For this review, take the finished solid that the model builds, in its own axes (mm). Coordinates: 2 decimals unless noted, no trailing zeros. Loops run counter-clockwise (first coordinate to the right, second up) from the corner with the lowest first, then second, coordinate; pieces in that order, holes last. Notation, with made-up numbers: (-9.5, -17) - (42.5, -17) arc R27 ccw to (42.5, 14) - close; hole circle Ø2 at (79.25, 4). An arc over 180 degrees is marked (long way). Use one line per item in the form item = value. Start each with the question number.
1. Add section C-C on z = 88.5. Give the boundary of the cut face in (x, y), and give its area (3 significant figures).
2. For pin 1 Ø10 at (x, y) = (-101, 20.5) entering from -Z; pin 2 Ø5 at (x, y) = (-81.5, 4.5) entering from -Z, all flat-tipped, find the tip position at first contact; note any pin that passes through.
3. To check wall thickness, follow probe 1 along X at (y, z) = (12.75, 77); probe 2 along X at (y, z) = (8.5, 27); probe 3 along Z at (x, y) = (-64.5, 15.5). State the ranges of each line that lie inside material, in increasing order.
4. Add section B-B on x = -157. Give the boundary of the cut face in (y, z), and give its area (3 significant figures).
5. Add section A-A on y = 8.5. Give the boundary of the cut face in (x, z), and give its area (3 significant figures).
```python
from build123d import *

# Parameters (mm, degrees)
EXTRUDE_1_DEPTH = 30


with BuildPart() as part:
    # 草图1 → 凸台-拉伸1 (new body)
    with BuildSketch(Plane(origin=(0, 0, 0), x_dir=(1, 0, 0), z_dir=(0, 1, 0))):
        Polygon((0, 0), (-30, 0), (-200, -98.149545762), (-200, -128.149545762), (-20, -128.149545762), (0, -108.149545762), align=None)
    extrude(amount=EXTRUDE_1_DEPTH)


solid = part.part
```
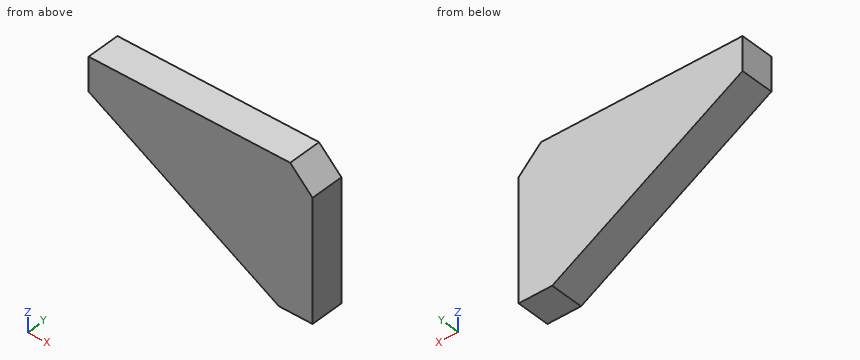
Conclusion:
q1.outline = (-183.29, 0) - (0, 0) - (0, 30) - (-183.29, 30) - close
q1.area = 5,500 mm^2
q2.pin_1 = 38.11
q2.pin_2 = 28.29
q3.probe_1 = -163.37 to 0
q3.probe_2 = -76.77 to 0
q3.probe_3 = 19.92 to 128.15
q4.outline = (0, 73.32) - (30, 73.32) - (30, 128.15) - (0, 128.15) - close
q4.area = 1,640 mm^2
q5.outline = (-200, 98.15) - (-30, 0) - (0, 0) - (0, 108.15) - (-20, 128.15) - (-200, 128.15) - close
q5.area = 17,100 mm^2
